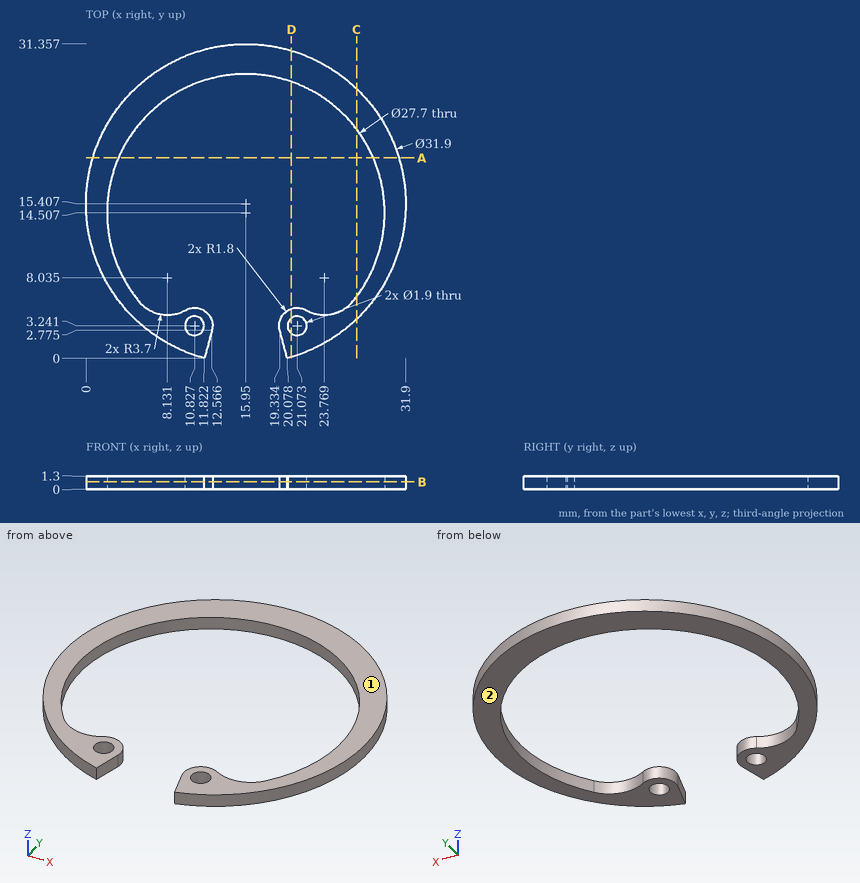
Design review of the part shown in the three views and the two pictorial views. Dimensions are in mm from the part's minimum x, y and z. Round coordinates to 2 decimals unless told otherwise and drop trailing zeros. Write each loop counter-clockwise with the first axis right and the second up, starting at its lowest first coordinate (ties: lowest second). Pieces come first, ordered by that corner, then holes. Notation, with made-up numbers: (-37.5, 37) - (0.5, 37) arc R19 cw to (0.5, 65) - close; hole circle Ø5 at (40, 89). An arc over 180 degrees is marked (long way). Write item = value, one per line. Start each with the question number.
1. Draft analysis for pull direction Z (two halves, no side actions). For the marked faces 1 and 2, state which applies: released by +Z, released by -Z, zero draft, split by the parting line, or undercut.
2. For pin 1 Ø8 at (x, y) = (21, 4) entering from -Z, flat-tipped, find the tip position at first contact; note if it passes through.
3. Consider section D-D on x = 20.5. State the section outline as (y, z) points.
4. Consider section B-B on z = 0.75. Give the number of separate pieces and of enclosed holes in the cut face, plus the area to 3 significant figures.
5. Wall thickness on L1, parallel to Y at x = 10, z = 0.45 (1 decimal); L2, parallel to Y at x = 21, z = 0.7 (1 decimal); L3, parallel to Y at x = 24.5, z = 1: over which ranges is each line inside the solid? List them lowest first.
6. Consider section A-A on y = 20. State the section outline as (x, z) points (1 decimal).
7. Consider section C-C on x = 27. State the section outline as (y, z) points (1 decimal).
Evaluation:
q1.face_1 = released by +Z
q1.face_2 = released by -Z
q2.pin_1 = 0
q3.outline = (0.12, 0) - (2.48, 0) - (2.48, 1.3) - (0.12, 1.3) - close; (4, 0) - (4.95, 0) - (4.95, 1.3) - (4, 1.3) - close; (27.59, 0) - (30.69, 0) - (30.69, 1.3) - (27.59, 1.3) - close
q4.separate_pieces = 1
q4.enclosed_holes = 2
q4.area = 208 mm2
q5.L1 = 0.6 to 2.8, 3.7 to 4.8, 27 to 30.2
q5.L2 = 0.3 to 2.3, 4.2 to 5, 27.4 to 30.5
q5.L3 = 1.94 to 4.41, 25.4 to 28.87
q6.outline = (0.7, 0) - (3.2, 0) - (3.2, 1.3) - (0.7, 1.3) - close; (28.7, 0) - (31.2, 0) - (31.2, 1.3) - (28.7, 1.3) - close
q7.outline = (3.9, 0) - (6.2, 0) - (6.2, 1.3) - (3.9, 1.3) - close; (22.9, 0) - (26.9, 0) - (26.9, 1.3) - (22.9, 1.3) - close
